Can you work these out from the model? Positions are in its coordinate system, mm. Face numbers are marked on the shaded views. A direction names the side the tool comes from. Coordinates: 2 decimals unless noted, no trailing zeros. Write each loop counter-clockwise with the first axis right and the second up, starting at its lowest first coordinate (ties: lowest second). Pieces come first, ordered by that corner, then holes. Notation, with made-up numbers: M 45.5,35 L 50.5,35 A23 ccw 50.5,50 Z; hole C 71.25,26.5 d8. An arc over 180 degrees is marked long. Answer as a JSON object with one key per item and string values. Group by question number.
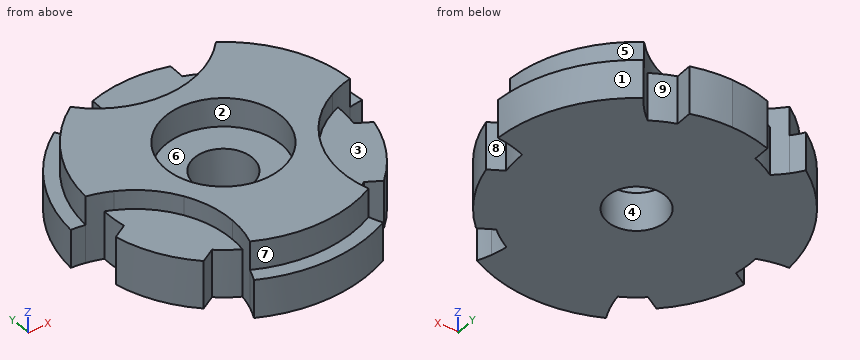
from build123d import *

# Parameters (mm, degrees)
BASE_DISC_SKETCH_R    = 75
BASE_DISC_DEPTH       = 20
HUB_BOSS_SKETCH_R     = 68
HUB_BOSS_DEPTH        = 15
LOBE_START            = -35
LOBE_RECESS_CUT_DEPTH = 35
COUPLING_LOBES_DEPTH  = 25
COUNTERBORE_SKETCH_R  = 30
COUNTERBORE_DEPTH     = 15
THROUGH_BORE_SKETCH_R = 15
THROUGH_BORE_DEPTH    = 20


with BuildPart() as part:
    # Base Disc Sketch → Base Disc (new body)
    with BuildSketch(Plane.XY):
        Circle(BASE_DISC_SKETCH_R)
    extrude(amount=BASE_DISC_DEPTH)

    # Hub Boss Sketch → Hub Boss (add)
    with BuildSketch(Plane.XY.offset(20)):
        Circle(HUB_BOSS_SKETCH_R)
    extrude(amount=HUB_BOSS_DEPTH)

    # Lobe Recess Sketch → Lobe Recess Cut (cut)
    with BuildSketch(Plane.XY.offset(35).offset(LOBE_START)):
        with BuildLine():
            ThreePointArc((-37.386628626, 56.8), (-19.514097468, 65.139849555), (0, 68))
            Line((0, 68), (0, 90))
            ThreePointArc((0, 90), (-25, 86.458082329), (-48.032267961, 76.111111111))
            ThreePointArc((-48.032267961, 76.111111111), (-43.787289555, 65.861373829), (-37.386628626, 56.8))
        make_face()
        with BuildLine():
            Line((0, 90), (0, 68))
            ThreePointArc((0, 68), (19.514097468, 65.139849555), (37.386628626, 56.8))
            ThreePointArc((37.386628626, 56.8), (43.787289555, 65.861373829), (48.032267961, 76.111111111))
            ThreePointArc((48.032267961, 76.111111111), (25, 86.458082329), (0, 90))
        make_face()
        with BuildLine():
            ThreePointArc((-37.386628626, 56.8), (-20.493901532, 44.392982996), (0, 40))
            Line((0, 40), (0, 68))
            ThreePointArc((0, 68), (-19.514097468, 65.139849555), (-37.386628626, 56.8))
        make_face()
        with BuildLine():
            Line((0, 68), (0, 40))
            ThreePointArc((0, 40), (20.493901532, 44.392982996), (37.386628626, 56.8))
            ThreePointArc((37.386628626, 56.8), (19.514097468, 65.139849555), (0, 68))
        make_face()
        with BuildLine():
            ThreePointArc((58.889727457, -34), (46.655715779, -49.469628917), (30.496928622, -60.777770152))
            ThreePointArc((30.496928622, -60.777770152), (35.143978087, -70.851592032), (41.898021752, -79.652719811))
            ThreePointArc((41.898021752, -79.652719811), (62.374895659, -64.879676259), (77.942286341, -45))
            Line((77.942286341, -45), (58.889727457, -34))
        make_face()
        with BuildLine():
            ThreePointArc((67.883557248, 3.977770152), (67.970883078, 1.989737061), (68, 0))
            ThreePointArc((68, 0), (65.682956188, -17.599695067), (58.889727457, -34))
            Line((58.889727457, -34), (77.942286341, -45))
            ThreePointArc((77.942286341, -45), (86.933324366, -23.293714059), (90, 0))
            ThreePointArc((90, 0), (89.982570741, 1.771147347), (89.930289713, 3.5416087))
            ThreePointArc((89.930289713, 3.5416087), (78.931267642, 4.990218203), (67.883557248, 3.977770152))
        make_face()
        with BuildLine():
            Line((68, 0), (56.147791623, 0))
            ThreePointArc((56.147791623, 0), (43.892842113, -8.385312403), (34.641016151, -20))
            Line((34.641016151, -20), (58.889727457, -34))
            ThreePointArc((58.889727457, -34), (65.682956188, -17.599695067), (68, 0))
        make_face()
        with BuildLine():
            Line((58.889727457, -34), (34.641016151, -20))
            ThreePointArc((34.641016151, -20), (28.198500258, -39.944730847), (30.496928622, -60.777770152))
            ThreePointArc((30.496928622, -60.777770152), (46.655715779, -49.469628917), (58.889727457, -34))
        make_face()
        with BuildLine():
            ThreePointArc((67.883557248, 3.977770152), (61.891970748, 2.353852741), (56.147791623, 0))
            Line((56.147791623, 0), (68, 0))
            ThreePointArc((68, 0), (67.970883078, 1.989737061), (67.883557248, 3.977770152))
        make_face()
        with BuildLine():
            ThreePointArc((-41.898021752, -79.652719811), (-35.143978087, -70.851592032), (-30.496928622, -60.777770152))
            ThreePointArc((-30.496928622, -60.777770152), (-46.655715779, -49.469628917), (-58.889727457, -34))
            Line((-58.889727457, -34), (-77.942286341, -45))
            ThreePointArc((-77.942286341, -45), (-62.374895659, -64.879676259), (-41.898021752, -79.652719811))
        make_face()
        with BuildLine():
            ThreePointArc((-58.889727457, -34), (-65.682956188, -17.599695067), (-68, 0))
            ThreePointArc((-68, 0), (-67.970883078, 1.989737061), (-67.883557248, 3.977770152))
            ThreePointArc((-67.883557248, 3.977770152), (-78.931267642, 4.990218203), (-89.930289713, 3.5416087))
            ThreePointArc((-89.930289713, 3.5416087), (-87.374895659, -21.57840607), (-77.942286341, -45))
            Line((-77.942286341, -45), (-58.889727457, -34))
        make_face()
        with BuildLine():
            ThreePointArc((-34.641016151, -20), (-43.892842113, -8.385312403), (-56.147791623, 0))
            Line((-56.147791623, 0), (-68, 0))
            ThreePointArc((-68, 0), (-65.682956188, -17.599695067), (-58.889727457, -34))
            Line((-58.889727457, -34), (-34.641016151, -20))
        make_face()
        with BuildLine():
            ThreePointArc((-27.942286341, -45), (-29.645995026, -32.059047745), (-34.641016151, -20))
            Line((-34.641016151, -20), (-58.889727457, -34))
            ThreePointArc((-58.889727457, -34), (-46.655715779, -49.469628917), (-30.496928622, -60.777770152))
            ThreePointArc((-30.496928622, -60.777770152), (-28.585078732, -52.99162418), (-27.942286341, -45))
        make_face()
        with BuildLine():
            Line((-68, 0), (-56.147791623, 0))
            ThreePointArc((-56.147791623, 0), (-61.891970748, 2.353852741), (-67.883557248, 3.977770152))
            ThreePointArc((-67.883557248, 3.977770152), (-67.970883078, 1.989737061), (-68, 0))
        make_face()
    extrude(amount=LOBE_RECESS_CUT_DEPTH, mode=Mode.SUBTRACT)

    # Coupling Lobes Sketch → Coupling Lobes (add)
    with BuildSketch(Plane(origin=(0, 0, 0), x_dir=(-1, 0, 0), z_dir=(0, 0, -1))):
        with BuildLine():
            ThreePointArc((-31.426968053, 51.111111111), (-16.666666667, 42.859547921), (0, 40))
            Line((0, 40), (0, 68))
            ThreePointArc((0, 68), (-10.112445497, 67.243872926), (-20, 64.992307237))
            Line((-20, 64.992307237), (-20, 56.568542495))
            ThreePointArc((-20, 56.568542495), (-25.857864376, 54.142135624), (-31.426968053, 51.111111111))
        make_face()
        with BuildLine():
            Line((0, 68), (0, 40))
            ThreePointArc((0, 40), (16.666666667, 42.859547921), (31.426968053, 51.111111111))
            ThreePointArc((31.426968053, 51.111111111), (25.857864376, 54.142135624), (20, 56.568542495))
            Line((20, 56.568542495), (20, 64.992307237))
            ThreePointArc((20, 64.992307237), (10.112445497, 67.243872926), (0, 68))
        make_face()
        with BuildLine():
            Line((-46.284989118, -49.816661694), (-38.989794856, -45.604779323))
            ThreePointArc((-38.989794856, -45.604779323), (-33.959532677, -49.464635249), (-28.550036612, -52.772108253))
            ThreePointArc((-28.550036612, -52.772108253), (-34.641016151, -20), (-59.977004664, 1.660997142))
            ThreePointArc((-59.977004664, 1.660997142), (-59.817397053, -4.677500374), (-58.989794856, -10.963763172))
            Line((-58.989794856, -10.963763172), (-66.284989118, -15.175645543))
            ThreePointArc((-66.284989118, -15.175645543), (-58.889727457, -34), (-46.284989118, -49.816661694))
        make_face()
        with BuildLine():
            Line((66.284989118, -15.175645543), (58.989794856, -10.963763172))
            ThreePointArc((58.989794856, -10.963763172), (59.817397053, -4.677500374), (59.977004664, 1.660997142))
            ThreePointArc((59.977004664, 1.660997142), (34.641016151, -20), (28.550036612, -52.772108253))
            ThreePointArc((28.550036612, -52.772108253), (33.959532677, -49.464635249), (38.989794856, -45.604779323))
            Line((38.989794856, -45.604779323), (46.284989118, -49.816661694))
            ThreePointArc((46.284989118, -49.816661694), (58.889727457, -34), (66.284989118, -15.175645543))
        make_face()
    extrude(amount=-COUPLING_LOBES_DEPTH)

    # Counterbore Sketch → Counterbore (cut)
    with BuildSketch(Plane.XY.offset(35)):
        Circle(COUNTERBORE_SKETCH_R)
    extrude(amount=-COUNTERBORE_DEPTH, mode=Mode.SUBTRACT)

    # Through Bore Sketch → Through Bore (cut)
    with BuildSketch(Plane.XY.offset(20)):
        Circle(THROUGH_BORE_SKETCH_R)
    extrude(amount=-THROUGH_BORE_DEPTH, mode=Mode.SUBTRACT)


solid = part.part
Q1. Please list where these lines run through material, in increasing order: L1, parallel to Z at x = -57.5, y = 40; L2, parallel to Z at x = 51, y = -29.5; L3, parallel to X at y = 58, z = 21.
Q2. We'd pull the mould along X, two halves only. Please class the marked faces 1, 2, 3 and 4: pulls with the +X half, pulls with the -X half, needs draft (parallel to the pull), parting line crosses it, or undercut.
Q3. If we section it at A-A on z = 4: List the corners of the cut face in (x, y) for me, and give its area (3 significant figures).
Q4. On a 3-axis mill with a long thin cutter (end or side, diameter ignored), from which of +Z, -Z, +X, -X, +Y, -Y can I reach the whole of each face in a straight line? I mean the marked faces 5, 6, 7, 8 and 9. Say none if no direction works.
Q5. If we section it at B-B on y = -56: List the corners of the cut face in (x, z) for me.
Q6. Will these pins go through, and if not, where does the flat tip stop? pin 1 (6.5 mm diameter, centred on y = 60, z = 9.5, fed in from -X); pin 2 (5 mm diameter, centred on x = -11, z = 31, fed in from +Y); pin 3 (9.5 mm diameter, centred on y = 61.5, z = 13, fed in from +X).
Reply:
{
 "1": {"L1": "0 to 20", "L2": "0 to 25", "L3": "-20 to 20"},
 "2": {"face 1": "pulls with the +X half", "face 2": "undercut", "face 3": "needs draft", "face 4": "undercut"},
 "3": {"outline": "M -74.84,4.9 A50 cw -59.98,1.66 A60 ccw -58.99,-10.96 L -66.28,-15.18 A68 ccw -46.28,-49.82 L -38.99,-45.6 A60 ccw -28.55,-52.77 A50 cw -33.17,-67.26 A75 ccw 33.17,-67.26 A50 cw 28.55,-52.77 A60 ccw 38.99,-45.6 L 46.28,-49.82 A68 ccw 66.28,-15.18 L 58.99,-10.96 A60 ccw 59.98,1.66 A50 cw 74.84,4.9 A75 ccw 41.67,62.36 A50 cw 31.43,51.11 A60 ccw 20,56.57 L 20,64.99 A68 ccw -20,64.99 L -20,56.57 A60 ccw -31.43,51.11 A50 cw -41.67,62.36 A75 ccw Z; hole C 0,0 d30", "area": "14,400 mm^2"},
 "4": {"face 5": "+Z, +X, +Y", "face 6": "+Z", "face 7": "+Z, -Y", "face 8": "+Z, -Z, +X", "face 9": "+Z, -Z, +Y"},
 "5": {"outline": "M -29.17,0 L 29.17,0 L 29.17,35 L -29.17,35 Z"},
 "6": {"pin 1": "x = -49.04", "pin 2": "y = 41.86", "pin 3": "x = 49.04"}
}
